Build history of the part. All positions in model axes, mm. Round coordinates to 2 decimals unless told otherwise and drop trailing zeros. Order: outer loops, then holes, each group sorted by start corner. A loop starts at its lowest first (then second) coordinate and runs counter-clockwise, first axis right, second up. Notation, with made-up numbers: M 72.25,45.5 L 128.25,45.5 A14 cw 128.25,59.5 Z; hole C 86,83.25 d2. An arc over 180 degrees is marked long. One line per item, written item: value. Start each with the question number.
Item 1: Probe L1, parallel to Z at x = -4.5, y = 1259; L2, parallel to X at y = 955.5, z = 22.5; L3, parallel to Y at x = 25.5, z = -25.5. List the from-to ranges inside material, lowest first.
Item 2: Band-saw the part on A-A, the plane y = 463. Write the cut outline in (x, z), then the cut area to 3 significant figures.
Item 3: Band-saw the part on B-B, the plane x = 1.5. Write the cut outline in (y, z).
```python
from build123d import *

# Parameters (mm, degrees)
GB_T_6728_2002_SQUARE_HOLLOW_SECTION_60_DEPTH = 1460
CUT_EXTRUDE1_DEPTH                            = 1462.5402834
CUT_EXTRUDE1_DEPTH_BACK                       = 1462.5402834


with BuildPart() as part:
    # Sketch1 → GB/T 6728-2002 square hollow section 60×60×4(1) (new body)
    with BuildSketch(Plane(origin=(0, 0, 0), x_dir=(-1, 0, 0), z_dir=(0, 1, 0))):
        with BuildLine():
            Line((-22, -30), (22, -30))
            ThreePointArc((22, -30), (27.656854249, -27.656854249), (30, -22))
            Line((30, -22), (30, 22))
            ThreePointArc((30, 22), (27.656854249, 27.656854249), (22, 30))
            Line((22, 30), (-22, 30))
            ThreePointArc((-22, 30), (-27.656854249, 27.656854249), (-30, 22))
            Line((-30, 22), (-30, -22))
            ThreePointArc((-30, -22), (-27.656854249, -27.656854249), (-22, -30))
        make_face()
        with BuildLine():
            Line((-22, -26), (22, -26))
            ThreePointArc((22, -26), (24.828427125, -24.828427125), (26, -22))
            Line((26, -22), (26, 22))
            ThreePointArc((26, 22), (24.828427125, 24.828427125), (22, 26))
            Line((22, 26), (-22, 26))
            ThreePointArc((-22, 26), (-24.828427125, 24.828427125), (-26, 22))
            Line((-26, 22), (-26, -22))
            ThreePointArc((-26, -22), (-24.828427125, -24.828427125), (-22, -26))
        make_face(mode=Mode.SUBTRACT)
    extrude(amount=GB_T_6728_2002_SQUARE_HOLLOW_SECTION_60_DEPTH)

    # Sketch2 → Cut-Extrude1 (cut, two sides: drawn at the far end of the back side and taken through both)
    with BuildSketch(Plane.XY.offset(30).offset(-CUT_EXTRUDE1_DEPTH_BACK)):
        Polygon((-30, 1460), (30, 1376.03139841), (30, 1460), align=None)
        Polygon((-30, 0), (-30, 83.96860159), (30, 0), align=None)
    extrude(amount=CUT_EXTRUDE1_DEPTH + CUT_EXTRUDE1_DEPTH_BACK, mode=Mode.SUBTRACT)


solid = part.part
```
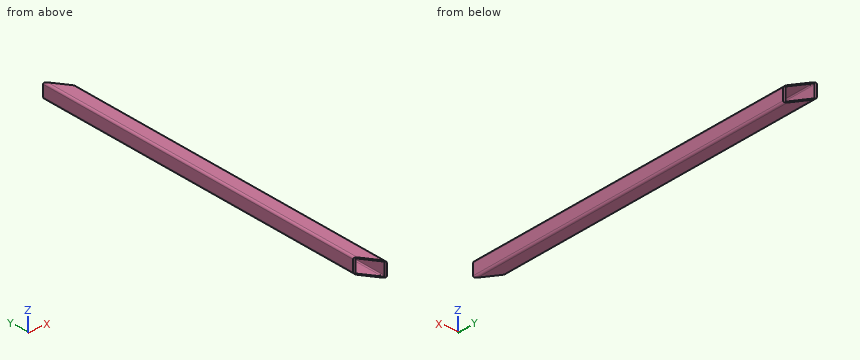
Output:
1. L1: z = -30 to -26, 26 to 30
1. L2: x = -29.98 to -25.97, 25.97 to 29.98
1. L3: y = 6.3 to 1382.33
2. outline: M -30,-22 A8 ccw -22,-30 L 22,-30 A8 ccw 30,-22 L 30,22 A8 ccw 22,30 L -22,30 A8 ccw -30,22 Z; hole M -26,-22 A4 ccw -22,-26 L 22,-26 A4 ccw 26,-22 L 26,22 A4 ccw 22,26 L -22,26 A4 ccw -26,22 Z
2. area: 855 mm²
3. outline: M 39.89,-30 L 1415.92,-30 L 1415.92,-26 L 39.89,-26 Z; M 39.89,26 L 1415.92,26 L 1415.92,30 L 39.89,30 Z
